The figure shows three views and two pictorial views of one solid part (mm, origin at its lowest corner). Answer the questions. A direction names the side the tool comes from. Coordinates: 2 decimals unless noted, no trailing zeros. Order: outer loops, then holes, each group sorted by start corner. A loop starts at its lowest first (then second) coordinate and runs counter-clockwise, first axis right, second up. Notation, with made-up numbers: (68.5, 38.25) -> (75.5, 38.25) arc R26 ccw to (75.5, 54.25) -> close; hole circle Ø1 at (52.25, 88.25). An arc over 180 degrees is marked (long way). Return JSON: item names as keys, results as strings.
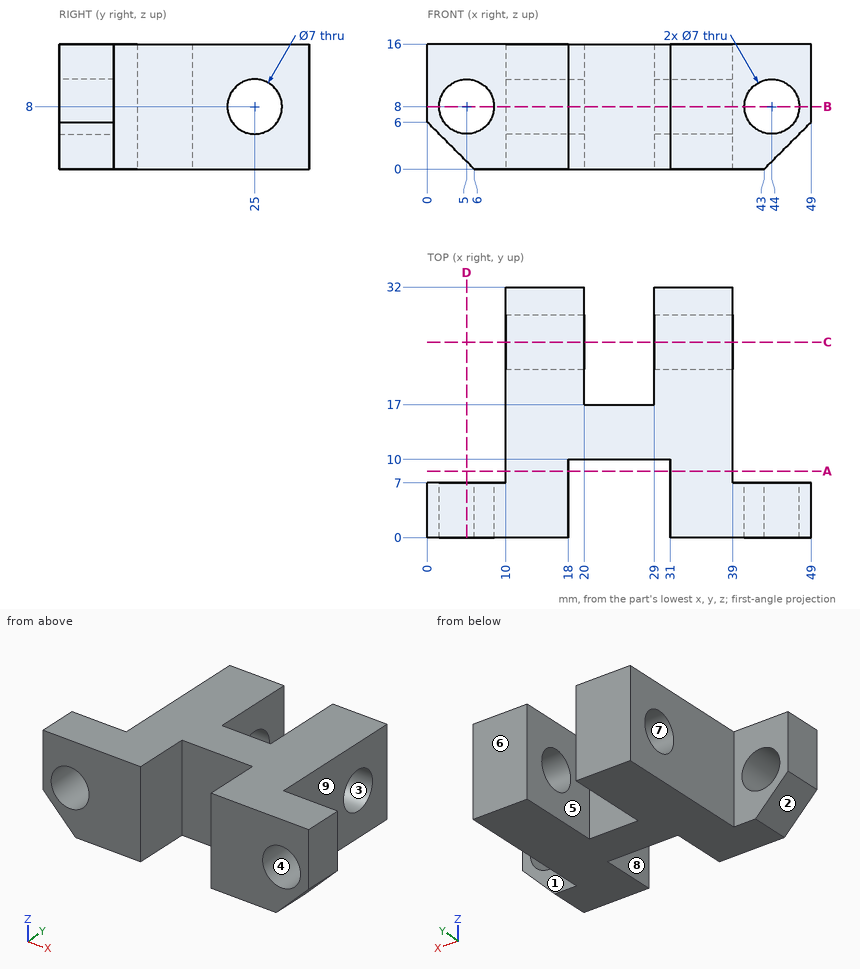
1. The part is cut by section D-D on x = 5. Give the vertices of the cut face in (y, z).
Answer block:
{"outline": "(0, 1) -> (7, 1) -> (7, 4.5) -> (0, 4.5) -> close; (0, 11.5) -> (7, 11.5) -> (7, 16) -> (0, 16) -> close"}
2. For the marked faces 5, 6, 7, 8 and 9, determine the directions among +Z, -Z, +X, -X, +Y, -Y from which every point of the face is accessible in a straight line to the end or side of a thin tool.
Answer block:
{"face 5": "+Z, -Z, +Y", "face 6": "+Z, -Z, +X, -X, +Y", "face 7": "+X, -X", "face 8": "+Z, -Z, -Y", "face 9": "+Z, -Z, +X, +Y"}
3. Each of these flat-tipped pins is pushed along its axis until it touches: pin 1 Ø1 at (x, z) = (8.5, 12) entering from -Y; pin 2 Ø8 at (y, z) = (18.5, 6) entering from -X; pin 3 Ø3 at (x, z) = (6.5, 7) entering from +Y; pin 4 Ø4 at (x, z) = (21.5, 6) entering from -Y. Where does it stop, or does it pass through?
Answer block:
{"pin 1": "stops at y = 0", "pin 2": "stops at x = 10", "pin 3": "passes through", "pin 4": "stops at y = 10"}
4. The part is cut by section C-C on y = 25. Give the vertices of the cut face in (x, z), and give its area (3 significant figures).
Answer block:
{"outline": "(10, 0) -> (20, 0) -> (20, 4.5) -> (10, 4.5) -> close; (10, 11.5) -> (20, 11.5) -> (20, 16) -> (10, 16) -> close; (29, 0) -> (39, 0) -> (39, 4.5) -> (29, 4.5) -> close; (29, 11.5) -> (39, 11.5) -> (39, 16) -> (29, 16) -> close", "area": "180 mm2"}
5. Determine the mould class of the marked faces 1, 2, 3 and 4 for opening direction Z: pulls with the +Z half, pulls with the -Z half, needs draft (parallel to the pull), parting line crosses it, or undercut.
Answer block:
{"face 1": "needs draft", "face 2": "pulls with the -Z half", "face 3": "undercut", "face 4": "undercut"}
6. The part is cut by section B-B on z = 8. Give the number of separate pieces and of enclosed holes in the cut face, and give its area (3 significant figures).
Answer block:
{"separate pieces": "5", "enclosed holes": "0", "area": "565 mm2"}
7. The part is cut by section A-A on y = 8.5. Give the vertices of the cut face in (x, z), and give its area (3 significant figures).
Answer block:
{"outline": "(10, 0) -> (18, 0) -> (18, 16) -> (10, 16) -> close; (31, 0) -> (39, 0) -> (39, 16) -> (31, 16) -> close", "area": "256 mm2"}
8. Consider line 1 (X direction, y = 1.75, z = 8); line 2 (Y direction, x = 36.5, z = 8); line 3 (X direction, y = 30, z = 14.25). Determine where each line is inside the solid, lowest interval first. Write a range as from..to.
Answer block:
{"line 1": "x = 0..1.5, 8.5..18, 31..40.5, 47.5..49", "line 2": "y = 0..21.5, 28.5..32", "line 3": "x = 10..20, 29..39"}
